Work out the finished part from the listing and answer in its coordinate system (mm). Coordinates: 2 decimals unless noted, no trailing zeros. Order: outer loops, then holes, each group sorted by start corner. A loop starts at its lowest first (then second) coordinate and runs counter-clockwise, first axis right, second up. Notation, with made-up numbers: M -10.5,2 L 0.5,2 A15 cw 0.5,28 Z; hole C -14,-37.75 d9. An arc over 180 degrees is marked long. Answer in a Markdown table with one row per item. Add a question column.
Item 1: The part is cut by section B-B (y = 317). Write down the section's boundary in (x, z), then the cut area to 3 significant figures.
Item 2: The part is cut by section C-C (x = 4.5). Write down the section's boundary in (y, z).
Item 3: Consider line 1 (Y direction, x = 30.5, z = 1.7); line 2 (Z direction, x = 27, y = 311.5); line 3 (Z direction, x = 21.5, y = 321). Determine where each line is inside the solid, lowest interval first. Write a range as from..to.
Item 4: The mould has two halves that part along X. Classify faces 1 (the face through (-13.96, 308.79, 2.59)), 2 (the face through (0.67, 298.39, 1.93)), 3 (the face through (11.4, 309.2, 2.9)): released by +X, released by -X, zero draft, split by the parting line, or undercut.
Item 5: The part is cut by section D-D (z = 2.5). State how many separate pieces and enclosed holes the cut face has, then the cut area to 3 significant figures.
Item 6: The part is cut by section A-A (y = 300.5). Write down the section's boundary in (x, z), then the cut area to 3 significant figures.
Item 7: Flat-ended cylindrical pins translate along their axes: pin 1 Ø5 at (x, y) = (17.5, 311.5) entering from -Z; pin 2 Ø1 at (x, y) = (4, 314.5) entering from +Z; pin 3 Ø1 at (y, z) = (305.5, 1) entering from +X. Find the tip coordinate at first contact, or state that the pin passes through.
from build123d import *

# Parameters (mm, degrees)
SKETCH1_W           = 50
SKETCH1_H           = 30
BOSS_EXTRUDE1_DEPTH = 3
M4_TAPPED_HOLE1_D   = 3.3
M3_TAPPED_HOLE1_D   = 2.5


with BuildPart() as part:
    # Sketch1 → Boss-Extrude1 (new body)
    with BuildSketch(Plane(origin=(18.523271638, 0, -0.440780543), x_dir=(-0.9988681377244376, 0, 0.04756514941544916), z_dir=(-0.04756514941544916, 0, -0.9988681377244377))):
        with Locations((7.591880235, 309)):
            Rectangle(SKETCH1_W, SKETCH1_H)
    extrude(amount=-BOSS_EXTRUDE1_DEPTH)

    # M4 Tapped Hole1 (through all)
    with Locations(Plane(origin=(0.020965792, 0, 0.44028164), x_dir=(-0.9988681377244376, 0, 0.04756514941544917), z_dir=(-0.047565149415449176, 0, -0.9988681377244377))):
        with Locations((-0.931391403, 320), (-0.931391403, 300)):
            Hole(M4_TAPPED_HOLE1_D / 2)

    # M3 Tapped Hole1 (through all)
    with Locations(Plane(origin=(0.020965792, 0, 0.44028164), x_dir=(-0.9988681377244376, 0, 0.04756514941544917), z_dir=(-0.047565149415449176, 0, -0.9988681377244377))):
        with Locations((-30.931391403, 322.2), (-30.931391403, 296.8)):
            Hole(M3_TAPPED_HOLE1_D / 2)


solid = part.part
Reply:
| question | item | result |
|---|---|---|
| 1 | outline | M -14.03,1.11 L 35.91,-1.27 L 36.05,1.73 L -13.89,4.11 Z |
| 1 | area | 150 mm2 |
| 2 | outline | M 294,0.23 L 324,0.23 L 324,3.23 L 294,3.23 Z |
| 3 | line 1 | y = 294..295.68, 297.92..321.08, 323.32..324 |
| 3 | line 2 | z = -0.84..2.16 |
| 3 | line 3 | z = -0.58..2.42 |
| 4 | face 1 | released by -X |
| 4 | face 2 | undercut |
| 4 | face 3 | released by +X |
| 5 | separate pieces | 1 |
| 5 | enclosed holes | 2 |
| 5 | area | 997 mm2 |
| 6 | outline | M -14.03,1.11 L -0.62,0.47 L -0.48,3.47 L -13.89,4.11 Z; M 2.52,0.32 L 35.91,-1.27 L 36.05,1.73 L 2.66,3.32 Z |
| 6 | area | 141 mm2 |
| 7 | pin 1 | stops at z = -0.51 |
| 7 | pin 2 | stops at z = 3.28 |
| 7 | pin 3 | stops at x = 36.04 |
